Here's the drawing with two shaded views (mm, measured from the low corner). I have some questions. Give positions to 0.01 mm unless a question says otherwise; leave off trailing zeros. Loops run counter-clockwise (first coordinate to the right, second up) from the corner with the lowest first, then second, coordinate; pieces in that order, holes last. Notation, with made-up numbers: (-22, 21.5) -> (28, 21.5) arc R20 ccw to (28, 50.5) -> close; hole circle Ø7 at (-27.75, -35). An arc over 180 degrees is marked (long way). Answer in a Markdown table with one row per item. Add a question column.
Item 1: If I drill on line 1 (Y direction, x = 57, z = 20.5); line 2 (X direction, y = 59.5, z = 23); line 3 (X direction, y = 71, z = 6), over which ranges is the centre line in solid material (lowest first)?
Item 2: If we section it at D-D (x = 16.5): Write out the boundary of the cut face in (y, z).
Item 3: We'd pull the mould along X, two halves only. Please class the marked faces 1, 2 and 3: released by +X, released by -X, zero draft, split by the parting line, or undercut.
Item 4: If we section it at A-A (y = 57): Write out the boundary of the cut face in (x, z), then the cut area to 3 significant figures.
Item 5: If we section it at C-C (z = 7.75): Write out the boundary of the cut face in (x, y).
Item 6: For P1, Ø1, axis at y = 101.5, z = 22.5, coming from the -X side, with a flat end and sliding along its axis, tell me the tip position at first contact or that it passes through.
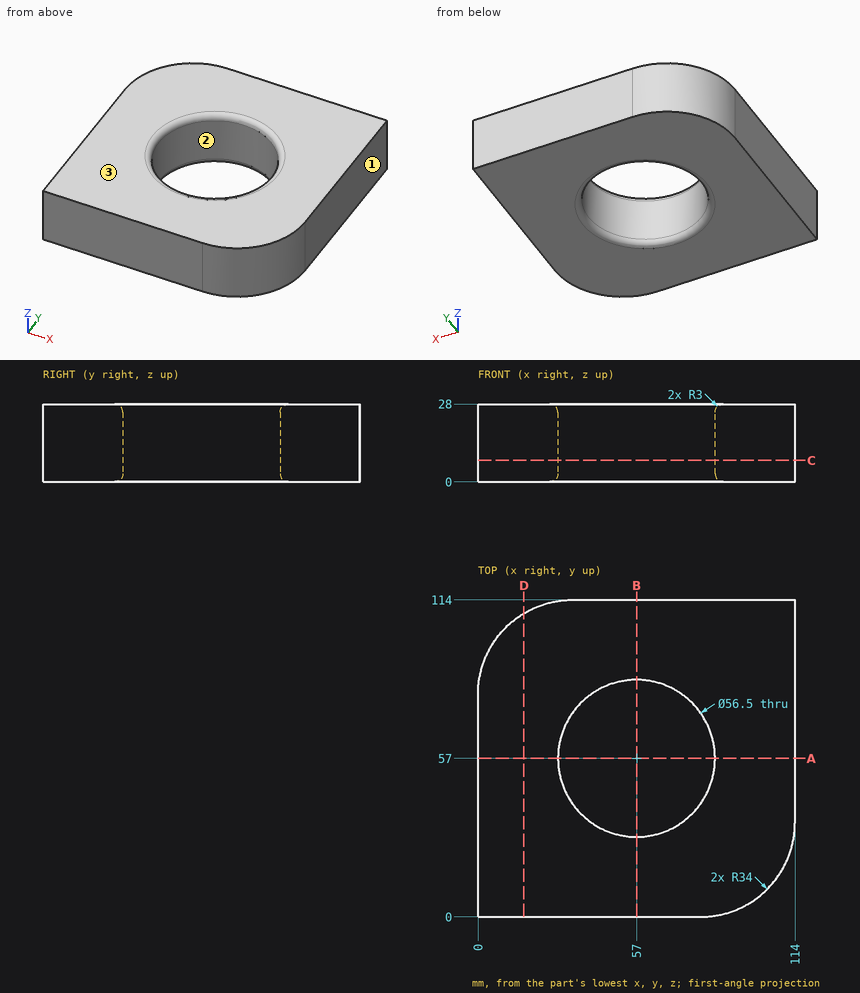
Recorded:
| question | item | result |
|---|---|---|
| 1 | line 1 | y = 0 to 28.75, 85.25 to 114 |
| 1 | line 2 | x = 0 to 28.86, 85.14 to 114 |
| 1 | line 3 | x = 0 to 32.46, 81.54 to 114 |
| 2 | outline | (0, 0) -> (109.15, 0) -> (109.15, 28) -> (0, 28) -> close |
| 3 | face 1 | released by +X |
| 3 | face 2 | undercut |
| 3 | face 3 | zero draft |
| 4 | outline | (0, 0) -> (25.75, 0) arc R3 ccw to (28.75, 3) -> (28.75, 25) arc R3 ccw to (25.75, 28) -> (0, 28) -> close; (85.25, 3) arc R3 ccw to (88.25, 0) -> (114, 0) -> (114, 28) -> (88.25, 28) arc R3 ccw to (85.25, 25) -> close |
| 4 | area | 1,600 mm^2 |
| 5 | outline | (0, 0) -> (80, 0) arc R34 ccw to (114, 34) -> (114, 114) -> (34, 114) arc R34 ccw to (0, 80) -> close; hole circle Ø56.5 at (57, 57) |
| 6 | P1 | stops at x = 7.26 |
